Source: CAD feature listing. Evaluate the final solid. Frame: model axes, mm. A direction names the side the tool comes from. Round coordinates to 2 decimals unless told otherwise and drop trailing zeros. Order: outer loops, then holes, each group sorted by start corner. A loop starts at its lowest first (then second) coordinate and runs counter-clockwise, first axis right, second up.
```python
from build123d import *

# Parameters (mm, degrees)
DISC_PROFILE_41_R         = 20.5
PORT_BLOCK_DISC_DEPTH     = 10
ARC_PORT_SLOTS_DEPTH      = 2.5
THROUGH_PORTS_PROFILE_R   = 2.5
THROUGH_PORTS_PROFILE_R_2 = 1
THROUGH_PORTS_DEPTH       = 32.5
PORT_POCKETS_PROFILE_R    = 2.5
PORT_POCKETS_DEPTH        = 5


with BuildPart() as part:
    # Disc Profile Ø41 → Port Block Disc (new body)
    with BuildSketch(Plane.XY):
        Circle(DISC_PROFILE_41_R)
    extrude(amount=PORT_BLOCK_DISC_DEPTH)

    # Arc Port Slots Profile → Arc Port Slots (cut)
    with BuildSketch(Plane.XY.offset(10)):
        with BuildLine():
            ThreePointArc((7.778174593, 7.778174593), (0, 11), (-7.778174593, 7.778174593))
            ThreePointArc((-7.778174593, 7.778174593), (-7.778174593, 3.535533906), (-3.535533906, 3.535533906))
            ThreePointArc((-3.535533906, 3.535533906), (0, 5), (3.535533906, 3.535533906))
            ThreePointArc((3.535533906, 3.535533906), (7.778174593, 3.535533906), (7.778174593, 7.778174593))
        make_face()
        with BuildLine():
            ThreePointArc((3.535533906, -3.535533906), (0, -5), (-3.535533906, -3.535533906))
            ThreePointArc((-3.535533906, -3.535533906), (-7.778174593, -3.535533906), (-7.778174593, -7.778174593))
            ThreePointArc((-7.778174593, -7.778174593), (0, -11), (7.778174593, -7.778174593))
            ThreePointArc((7.778174593, -7.778174593), (7.778174593, -3.535533906), (3.535533906, -3.535533906))
        make_face()
    extrude(amount=-ARC_PORT_SLOTS_DEPTH, mode=Mode.SUBTRACT)

    # Through Ports Profile → Through Ports (cut)
    with BuildSketch(Plane.XY.offset(10)):
        Circle(THROUGH_PORTS_PROFILE_R)
        with Locations((0, 8)):
            Circle(THROUGH_PORTS_PROFILE_R_2)
        with Locations((0, -8)):
            Circle(THROUGH_PORTS_PROFILE_R_2)
    extrude(amount=-THROUGH_PORTS_DEPTH, mode=Mode.SUBTRACT)

    # Port Pockets Profile → Port Pockets (cut)
    with BuildSketch(Plane(origin=(0, 0, 0), x_dir=(-1, 0, 0), z_dir=(0, 0, -1))):
        with Locations((12.5, 0)):
            Circle(PORT_POCKETS_PROFILE_R)
        with Locations((-12.5, 0)):
            Circle(PORT_POCKETS_PROFILE_R)
    extrude(amount=-PORT_POCKETS_DEPTH, mode=Mode.SUBTRACT)


solid = part.part
```
1. Pull-direction query (Y, two-part tool) for faces 1 (the face through (-4.444, -20.013, 4.93)), 2 (the face through (4, 0, 0)), 3 (the face through (0, -5, 9)); classes: released by +Y, released by -Y, zero draft, split by the parting line, or undercut.
2. Section D-D on x = -11.5. Return loops of the section in (y, z).
3. Line query: line 1 along Y through (x, z) = (0, 2); line 2 along Y through (x, z) = (-4.5, 9.5); line 3 along X through (y, z) = (-9, 9.5). Output: solid intervals per line, ascending.
4. First-contact query: pin 1 (3 mm diameter, centred on x = -12.5, y = 0, fed in from -Z); pin 2 (5 mm diameter, centred on x = -15.5, z = 6.5, fed in from -Y); pin 3 (2.5 mm diameter, centred on x = 0, y = 8, fed in from +Z); pin 4 (9 mm diameter, centred on x = 2.5, y = -6, fed in from +Z). Flat tips, straight axial feed; report the tip coordinate or a pass-through.
5. Section C-C on z = 3. Return loops of the section in (x, y).
6. Section A-A on y = 0. Return loops of the section in (x, z).
7. Access query for faces 4 (the face through (13, 0, 5)), 5 (the face through (0, 9, 4)), 6 (the face through (0, -11, 9)). Directions: +Z, -Z, +X, -X, +Y, -Y. A direction counts if a zero-diameter tool reaches every point of the face in a straight line with its end or side. Return the directions, or none.
8. Section B-B on x = 0. Return loops of the section in (y, z), plus the area to 3 significant figures.
Result:
1. face 1: split by the parting line
1. face 2: zero draft
1. face 3: undercut
2. outline: (-16.97, 0) - (-2.29, 0) - (-2.29, 5) - (2.29, 5) - (2.29, 0) - (16.97, 0) - (16.97, 10) - (-16.97, 10) - close
3. line 1: y = -20.5 to -9, -7 to -2.5, 2.5 to 7, 9 to 20.5
3. line 2: y = -20 to -10.04, -2.89 to 2.89, 10.04 to 20
3. line 3: x = -18.42 to -6.32, 6.32 to 18.42
4. pin 1: stops at z = 5
4. pin 2: stops at y = -15.85
4. pin 3: stops at z = 7.5
4. pin 4: stops at z = 10
5. outline: circle Ø41 at (0, 0); hole circle Ø5 at (-12.5, 0); hole circle Ø5 at (0, 0); hole circle Ø2 at (0, -8); hole circle Ø2 at (0, 8); hole circle Ø5 at (12.5, 0)
6. outline: (-20.5, 0) - (-15, 0) - (-15, 5) - (-10, 5) - (-10, 0) - (-2.5, 0) - (-2.5, 10) - (-20.5, 10) - close; (2.5, 0) - (10, 0) - (10, 5) - (15, 5) - (15, 0) - (20.5, 0) - (20.5, 10) - (2.5, 10) - close
7. face 4: -Z
7. face 5: +Z, -Z
7. face 6: +Z
8. outline: (-20.5, 0) - (-9, 0) - (-9, 7.5) - (-11, 7.5) - (-11, 10) - (-20.5, 10) - close; (-7, 0) - (-2.5, 0) - (-2.5, 10) - (-5, 10) - (-5, 7.5) - (-7, 7.5) - close; (2.5, 0) - (7, 0) - (7, 7.5) - (5, 7.5) - (5, 10) - (2.5, 10) - close; (9, 0) - (20.5, 0) - (20.5, 10) - (11, 10) - (11, 7.5) - (9, 7.5) - close
8. area: 300 mm2
